Verification items for this drawing (mm, ordinates from the low corner). A direction names the side the tool comes from. Round coordinates to 2 decimals unless told otherwise and drop trailing zeros. Loops run counter-clockwise (first coordinate to the right, second up) from the corner with the lowest first, then second, coordinate; pieces in that order, holes last. Notation, with made-up numbers: M 28,-36 L 65,-36 A18 cw 65,-14 Z; hole C 13,46.25 d8. An arc over 180 degrees is marked long. One line per item, written item: value.
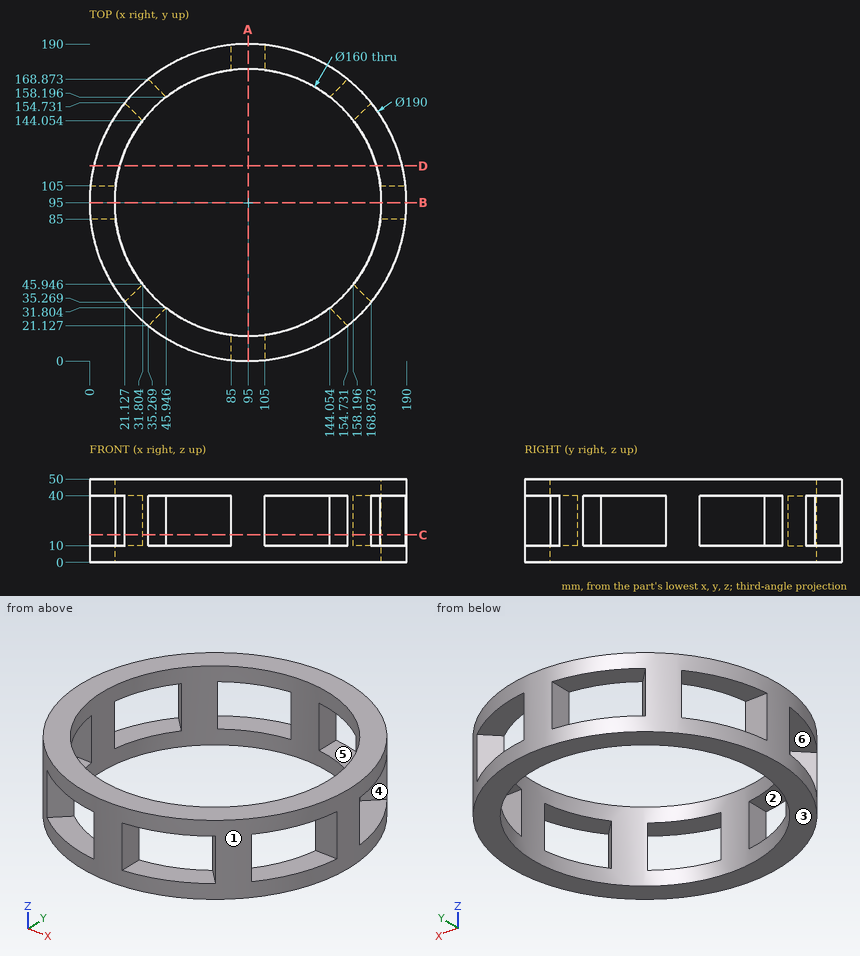
(1) Depth check by flat-ended pin: pin 1 Ø3 at (y, z) = (140.5, 44) entering from +X; pin 2 Ø7.5 at (y, z) = (6.5, 27) entering from +X; pin 3 Ø7.5 at (x, z) = (185.5, 21) entering from -Y; pin 4 Ø25 at (x, y) = (130, 14.5) entering from -Z. Enter the tip coordinate at first touch or a pass-through.
Completed:
pin 1: stops at x = 179.2
pin 2: stops at x = 105
pin 3: stops at y = 85
pin 4: stops at z = 0
(2) Sectioned sample at D-D on y = 117. Enter the section's corners in (x, z), and give its area (3 significant figures).
Completed:
outline: M 2.58,0 L 18.08,0 L 18.08,10 L 2.58,10 Z; M 2.58,40 L 18.08,40 L 18.08,50 L 2.58,50 Z; M 171.92,0 L 187.42,0 L 187.42,10 L 171.92,10 Z; M 171.92,40 L 187.42,40 L 187.42,50 L 171.92,50 Z
area: 620 mm^2
(3) Thickness scan on L1, parallel to Z at x = 75, y = 12.5; L2, parallel to Y at x = 95, z = 13; L3, parallel to X at y = 12, z = 34.5. Record the ranges inside material, lowest first. Write a range as from..to.
Completed:
L1: z = 0..10, 40..50
L2: y = 0..15, 175..190
L3: x = 85..105
(4) Sectioned sample at A-A on x = 95. Enter the section's corners in (y, z), and give its area (3 significant figures).
Completed:
outline: M 0,0 L 15,0 L 15,50 L 0,50 Z; M 175,0 L 190,0 L 190,50 L 175,50 Z
area: 1,500 mm^2
(5) Sectioned sample at C-C on z = 16.5. Count the separate pieces of the cut face and the enclosed holes in it, and give its area (3 significant figures).
Completed:
separate pieces: 8
enclosed holes: 0
area: 2,410 mm^2
(6) Tool access check on the marked faces 4, 5 and 6. Record the directions out of +Z, -Z, +X, -X, +Y, -Y that give a thin tool (end or side, any length) a straight path to the whole face; none if there is none.
Completed:
face 4: +X
face 5: +Y
face 6: -X
(7) Mould release check, pull along X, two halves, no side actions. Record for the marked faces 1, 2 and 3: +X half, -X half, draft (parallel to the pull), parting line (faces both ways), or undercut.
Completed:
face 1: parting line
face 2: undercut
face 3: draft
